Can you work these out from the drawing? Everything is in mm from the part's minimum corner. A direction names the side the tool comes from. Round coordinates to 2 decimals unless told otherwise and drop trailing zeros. Write each loop counter-clockwise with the first axis right and the second up, starting at its lowest first coordinate (ties: lowest second). Pieces come first, ordered by that corner, then holes. Notation, with made-up numbers: (64.25, -29.75) -> (98.25, -29.75) arc R31 ccw to (98.25, -4.75) -> close; hole circle Ø1 at (82.25, 76). An arc over 180 degrees is marked (long way). Put each result on its own line as item: value. Start each with the question number.
1. Suppose I cut it at D-D (y = 1.25). Please give me the cut outline in (x, z), then the cut area to 3 significant figures.
2. Suppose I cut it at C-C (x = 10.75). Please give me the cut outline in (y, z), then the cut area to 3 significant figures.
3. Which directions (+Z, -Z, +X, -X, +Y, -Y) give clear straight access to the entire face, cutting with the end or side of a thin tool? Please do the marked faces 4, 5 and 6.
4. We'd pull the mould along X, two halves only. Please class the marked faces 1, 2 and 3: +X half, -X half, draft (parallel to the pull), parting line (faces both ways), or undercut.
5. Suppose I cut it at B-B (y = 3.8). Please give me the cut outline in (x, z), then the cut area to 3 significant figures.
6. Suppose I cut it at A-A (z = 4). Please give me the cut outline in (x, y).
7. For pin 1 (1.5 mm diameter, centred on x = 5.5, y = 3, fed in from +Z); pin 2 (2 mm diameter, centred on x = 18, y = 5.5, fed in from -Z); pin 3 (2.5 mm diameter, centred on x = 6, z = 4, fed in from -Y), each with a flat end and sliding along its axis, tell me the tip position at first contact or that it passes through.
8. I need wall thicknesses on probe 1 along Y at (x, z) = (22.5, 3.5); probe 2 along Z at (x, y) = (1.5, 5.2); probe 3 along X at (y, z) = (3.75, 3.5). Which ranges of each line are inside material? Lowest first, please. Write a range as from..to.
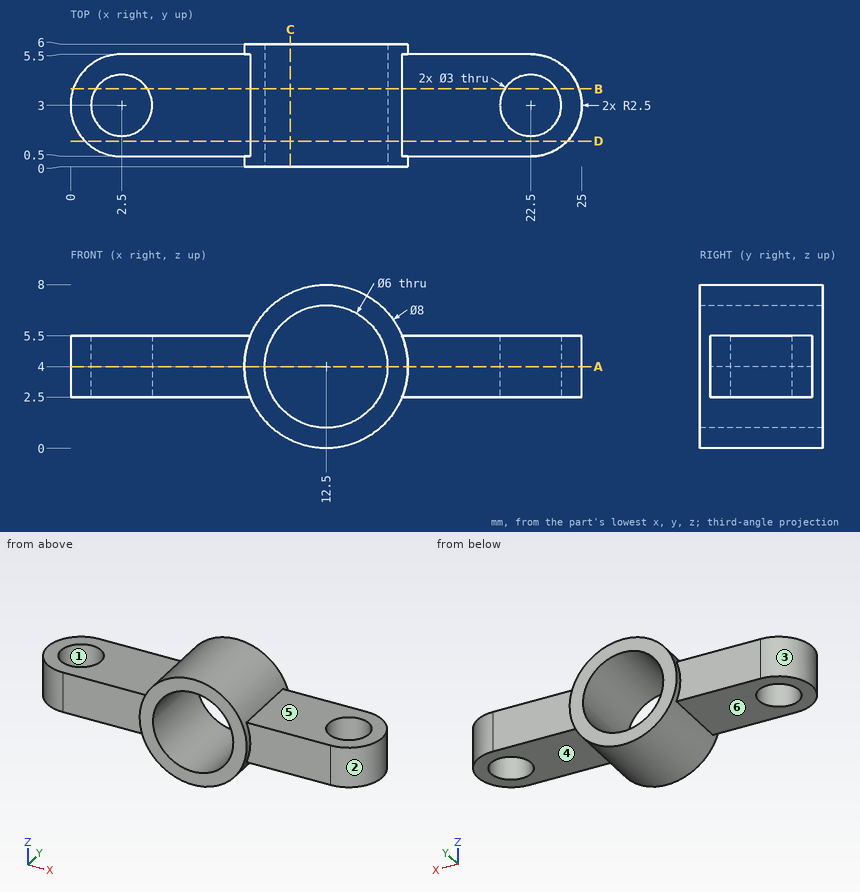
Verdict:
1. outline: (0.71, 2.5) -> (8.79, 2.5) arc R4 ccw to (16.21, 2.5) -> (24.29, 2.5) -> (24.29, 5.5) -> (16.21, 5.5) arc R4 ccw to (8.79, 5.5) -> (0.71, 5.5) -> close; hole circle Ø6 at (12.5, 4)
1. area: 69.3 mm^2
2. outline: (0, 0.4) -> (6, 0.4) -> (6, 1.56) -> (0, 1.56) -> close; (0, 6.44) -> (6, 6.44) -> (6, 7.6) -> (0, 7.6) -> close
2. area: 13.9 mm^2
3. face 4: -Z, +X, +Y, -Y
3. face 5: +Z, +X, +Y, -Y
3. face 6: -Z, -X, +Y, -Y
4. face 1: undercut
4. face 2: +X half
4. face 3: -X half
5. outline: (0.13, 2.5) -> (1.23, 2.5) -> (1.23, 5.5) -> (0.13, 5.5) -> close; (3.77, 2.5) -> (8.79, 2.5) arc R4 ccw to (16.21, 2.5) -> (21.23, 2.5) -> (21.23, 5.5) -> (16.21, 5.5) arc R4 ccw to (8.79, 5.5) -> (3.77, 5.5) -> close; (23.77, 2.5) -> (24.87, 2.5) -> (24.87, 5.5) -> (23.77, 5.5) -> close; hole circle Ø6 at (12.5, 4)
5. area: 57.6 mm^2
6. outline: (2.5, 0.5) -> (8.5, 0.5) -> (8.5, 0) -> (9.5, 0) -> (9.5, 6) -> (8.5, 6) -> (8.5, 5.5) -> (2.5, 5.5) arc R2.5 ccw to start; (15.5, 0) -> (16.5, 0) -> (16.5, 0.5) -> (22.5, 0.5) arc R2.5 ccw to (22.5, 5.5) -> (16.5, 5.5) -> (16.5, 6) -> (15.5, 6) -> close; hole circle Ø3 at (2.5, 3); hole circle Ø3 at (22.5, 3)
7. pin 1: stops at z = 5.5
7. pin 2: stops at z = 2.5
7. pin 3: stops at y = 0.5
8. probe 1: y = 0.5..1.5, 4.5..5.5
8. probe 2: z = 2.5..5.5
8. probe 3: x = 0.12..1.2, 3.8..9.54, 15.46..21.2, 23.8..24.88
